Verification items for the finished model (mm, model axes). A direction names the side the tool comes from. Coordinates: 2 decimals unless noted, no trailing zeros. Order: outer loops, then holes, each group sorted by start corner. A loop starts at its lowest first (then second) coordinate and runs counter-clockwise, first axis right, second up. Notation, with made-up numbers: M -31,53.5 L -8,53.5 A12 cw -8,68.5 Z; hole C -34,82.25 d1. An arc over 180 degrees is marked long. Return JSON: item names as keys, results as strings.
```python
from build123d import *

# Parameters (mm, degrees)
BOSS_EXTRUDE1_DEPTH = 160
SKETCH2_R           = 3
CUT_EXTRUDE1_DEPTH  = 8


with BuildPart() as part:
    # Sketch1 → Boss-Extrude1 (new body)
    with BuildSketch(Plane.XY):
        with BuildLine():
            Line((0, 0), (0, -137.894354723))
            ThreePointArc((0, -137.894354723), (4.778219722, -147.477980843), (15.30764827, -149.429495074))
            Line((15.30764827, -149.429495074), (231.30764827, -87.49249175))
            ThreePointArc((231.30764827, -87.49249175), (237.583626121, -83.179131677), (240, -75.957351399))
            Line((240, -75.957351399), (240, 0))
            Line((240, 0), (234, 0))
            Line((234, 0), (234, -75.957351399))
            ThreePointArc((234, -75.957351399), (232.79181306, -79.568241538), (229.653824135, -81.724921574))
            Line((229.653824135, -81.724921574), (13.653824135, -143.661924898))
            ThreePointArc((13.653824135, -143.661924898), (8.389109861, -142.686167783), (6, -137.894354723))
            Line((6, -137.894354723), (6, 0))
            Line((6, 0), (0, 0))
        make_face()
    extrude(amount=BOSS_EXTRUDE1_DEPTH)

    # Sketch2 → Cut-Extrude1 (cut)
    with BuildSketch(Plane(origin=(40.755797191, -142.132355795, 0), x_dir=(0.9612616959383188, 0.2756373558169997, 0), z_dir=(0.27563735581699966, -0.9612616959383187, 0))):
        with Locations((1.601767174, 140)):
            Circle(SKETCH2_R)
        with Locations((1.601767174, 20)):
            Circle(SKETCH2_R)
        with Locations((161.601767174, 140)):
            Circle(SKETCH2_R)
        with Locations((161.601767174, 20)):
            Circle(SKETCH2_R)
    extrude(amount=-CUT_EXTRUDE1_DEPTH, mode=Mode.SUBTRACT)


solid = part.part
```
Q1. Cross-section at B-B, the plane z = 114. Record the boundary of the cut face in (x, y), and give its area (3 significant figures).
Values:
{"outline": "M 0,-137.89 A12 ccw 15.31,-149.43 L 231.31,-87.49 A12 ccw 240,-75.96 L 240,0 L 234,0 L 234,-75.96 A6 cw 229.65,-81.72 L 13.65,-143.66 A6 cw 6,-137.89 L 6,0 L 0,0 Z", "area": "2,800 mm^2"}
Q2. Cross-section at A-A, the plane y = -11. Record the boundary of the cut face in (x, z), and give its area (3 significant figures).
Values:
{"outline": "M 0,0 L 6,0 L 6,160 L 0,160 Z; M 234,0 L 240,0 L 240,160 L 234,160 Z", "area": "1,920 mm^2"}
Q3. Cross-section at C-C, the plane y = -129. Record the boundary of the cut face in (x, z), and give its area (3 significant figures).
Values:
{"outline": "M 0,0 L 6,0 L 6,160 L 0,160 Z; M 64.79,0 L 86.55,0 L 86.55,160 L 64.79,160 Z", "area": "4,440 mm^2"}
Q4. Draft check along Z on faces 1 (the face through (119.4, -113.5, 0)), 2 (the face through (234, -37, 79)), 3 (the face through (196.83, -94.3, 142.53)). Enter one of: pulls with the +Z half, pulls with the -Z half, needs draft (parallel to the pull), parting line crosses it, or undercut.
Values:
{"face 1": "pulls with the -Z half", "face 2": "needs draft", "face 3": "undercut"}
Q5. Material ranges on line 1 along X through (y, z) = (-25.5, 104.5); line 2 along Y through (x, z) = (26.5, 151); line 3 along Y through (x, z) = (44, 23.5), recorded low to high.
Values:
{"line 1": "0 to 6, 234 to 240", "line 2": "-146.22 to -139.98", "line 3": "-141.2 to -134.96"}
Q6. Cross-section at D-D, the plane x = 188. Record the boundary of the cut face in (y, z).
Values:
{"outline": "M -99.91,0 L -93.67,0 L -93.67,160 L -99.91,160 Z"}
Q7. Go/stop test with flat-tipped pins: pin 1 (2 mm diameter, centred on x = 140, z = 78.5, fed in from +Y); pin 2 (12 mm diameter, centred on x = 80.5, z = 77.5, fed in from -Y); pin 3 (5 mm diameter, centred on x = 144.5, z = 113.5, fed in from -Y). Record where each tip stops, or that it passes through.
Values:
{"pin 1": "y = -107.15", "pin 2": "y = -132.46", "pin 3": "y = -113.1"}
Q8. Tool access check on faces 4 (the face through (232.824, -79.525, 78.88)), 5 (the face through (119.4, -113.5, 160)). Record the directions out of +Z, -Z, +X, -X, +Y, -Y that give a thin tool (end or side, any length) a straight path to the whole face; none if there is none.
Values:
{"face 4": "+Z, -Z, +Y", "face 5": "+Z, +X, -X, +Y, -Y"}
